from build123d import *

# Parameters (mm, degrees)
SKETCH_1_R          = 15
SKETCH_1_R_2        = 7.5
EXTRUDE_1_DEPTH     = 7
CUT_EXTRUDE_START   = -4
SKETCH_2_R          = 15
CUT_EXTRUDE_2_DEPTH = 4


with BuildPart() as part:
    # 草图1 → 凸台-拉伸1 (new body)
    with BuildSketch(Plane.XY):
        Circle(SKETCH_1_R)
        Circle(SKETCH_1_R_2, mode=Mode.SUBTRACT)
    extrude(amount=EXTRUDE_1_DEPTH)

    # 草图2 → 切除-拉伸2 (cut)
    with BuildSketch(Plane.XY.offset(7).offset(CUT_EXTRUDE_START)):
        Circle(SKETCH_2_R)
        with BuildLine():
            Line((-5.678908346, 10), (5.678908346, 10))
            ThreePointArc((5.678908346, 10), (0, -11.5), (-5.678908346, 10))
        make_face(mode=Mode.SUBTRACT)
    extrude(amount=CUT_EXTRUDE_2_DEPTH, mode=Mode.SUBTRACT)


solid = part.part
Geometry check sheet. Reference: the model listing, model coordinates, mm. Give positions to 0.01 mm unless a question says otherwise; leave off trailing zeros. Order: outer loops, then holes, each group sorted by start corner. A loop starts at its lowest first (then second) coordinate and runs counter-clockwise, first axis right, second up.
1. Scan lines: line 1 (Z direction, x = -12.25, y = -7.25); line 2 (Y direction, x = 1.75, z = 1.5); line 3 (X direction, y = 5.5, z = 4.75). Record each from-to range of solid material in increasing order.
Completed:
line 1: z = 0 to 3
line 2: y = -14.9 to -7.29, 7.29 to 14.9
line 3: x = -10.1 to -5.1, 5.1 to 10.1
2. Depth check by flat-ended pin: pin 1 (12 mm diameter, centred on x = 0, y = 0, fed in from +Z); pin 2 (1.5 mm diameter, centred on x = -6, z = 2, fed in from +Y); pin 3 (1 mm diameter, centred on x = -10, y = 8, fed in from +Z). Enter the tip coordinate at first touch or a pass-through.
Completed:
pin 1: passes through
pin 2: stops at y = 14.05
pin 3: stops at z = 3
3. Sectioned sample at C-C (z = 4). Record the boundary of the cut face in (x, y).
Completed:
outline: (-5.68, 10) arc R11.5 ccw (long way) to (5.68, 10) - close; hole circle Ø15 at (0, 0)
4. Sectioned sample at A-A (x = 0). Record the boundary of the cut face in (y, z), then the cut area to 3 significant figures.
Completed:
outline: (-15, 0) - (-7.5, 0) - (-7.5, 7) - (-11.5, 7) - (-11.5, 3) - (-15, 3) - close; (7.5, 0) - (15, 0) - (15, 3) - (10, 3) - (10, 7) - (7.5, 7) - close
area: 71.0 mm2
5. Draft check along Y on faces 1 (the face through (0, 10, 5)), 2 (the face through (0.423, -11.492, 4.972)), 3 (the face through (-7.493, 0.33, 3.451)), 4 (the face through (-0.2, 10.2, 3)). Enter one of: pulls with the +Y half, pulls with the -Y half, needs draft (parallel to the pull), parting line crosses it, or undercut.
Completed:
face 1: pulls with the +Y half
face 2: parting line crosses it
face 3: undercut
face 4: needs draft
6. Sectioned sample at B-B (y = 0). Record the boundary of the cut face in (x, z), then the cut area to 3 significant figures.
Completed:
outline: (-15, 0) - (-7.5, 0) - (-7.5, 7) - (-11.5, 7) - (-11.5, 3) - (-15, 3) - close; (7.5, 0) - (15, 0) - (15, 3) - (11.5, 3) - (11.5, 7) - (7.5, 7) - close
area: 77.0 mm2
7. Sectioned sample at D-D (x = -10.5). Record the boundary of the cut face in (y, z), then the cut area to 3 significant figures.
Completed:
outline: (-10.71, 0) - (10.71, 0) - (10.71, 3) - (4.69, 3) - (4.69, 7) - (-4.69, 7) - (-4.69, 3) - (-10.71, 3) - close
area: 102 mm2
